Geometry: final body of the model. Coordinates: model frame, mm. A direction names the side the tool comes from. Round coordinates to 2 decimals unless told otherwise and drop trailing zeros. Loops run counter-clockwise (first coordinate to the right, second up) from the corner with the lowest first, then second, coordinate; pieces in that order, holes last. Notation, with made-up numbers: M -10,-8.75 L 14,-8.75 A21 cw 14,15.25 Z; hole C 82.5,67.5 d10. An arc over 180 degrees is marked long. Answer as a JSON object with one key per item and string values.
```python
from build123d import *

# Parameters (mm, degrees)
CHAMFER1_SIZE         = 1.2
M3_TAPPED_HOLE1_D     = 2.5
M3_TAPPED_HOLE1_DEPTH = 7.5
M3_TAPPED_HOLE1_TIP   = 0.751075774
CHAMFER2_SIZE         = 0.5


with BuildPart() as part:
    # Sketch1 → Revolve1 (revolve)
    with BuildSketch(Plane.XY, mode=Mode.PRIVATE) as revolve1_sk:
        Polygon((0, 0), (0, 3), (2.5, 3), (2.5, 5), (5, 5), (5, 3), (10, 3), (10, 2.9), (55.5, 2.9), (55.5, 3), (65.5, 3), (65.5, 0), align=None)
    revolve(revolve1_sk.sketch.rotate(Axis((0, 0, 0), (1, 0, 0)), 90), axis=Axis((0, 0, 0), (1, 0, 0)))

    # Chamfer1
    chamfer1_edges = [part.edges().sort_by_distance(p)[0] for p in [
        (5, 0, -5),
    ]]
    chamfer(chamfer1_edges, length=CHAMFER1_SIZE)

    # M3 Tapped Hole1
    with Locations(Plane.ZY):
        with Locations((0, 0)):
            Hole(M3_TAPPED_HOLE1_D / 2, depth=M3_TAPPED_HOLE1_DEPTH)
            with Locations((0, 0, -(M3_TAPPED_HOLE1_DEPTH + M3_TAPPED_HOLE1_TIP / 2))):  # 118° drill point
                Cone(0, M3_TAPPED_HOLE1_D / 2, M3_TAPPED_HOLE1_TIP, mode=Mode.SUBTRACT)

    # Chamfer2
    chamfer2_edges = [part.edges().sort_by_distance(p)[0] for p in [
        (0, 0, -3),
        (65.5, 0, -3),
    ]]
    chamfer(chamfer2_edges, length=CHAMFER2_SIZE)


solid = part.part
```
1) First-contact query: pin 1 (6 mm diameter, centred on x = 42, y = -1, fed in from +Z); pin 2 (2 mm diameter, centred on y = -0.5, z = -3.5, fed in from +X); pin 3 (2 mm diameter, centred on x = 8, z = -1.5, fed in from +Y). Flat tips, straight axial feed; report the tip coordinate or a pass-through.
Geometry results:
{"pin 1": "z = 2.9", "pin 2": "x = 65.46", "pin 3": "y = 2.96"}
2) Cut plane A-A on x = 26. Return the cut outline in (y, z), and give its area (3 significant figures).
Geometry results:
{"outline": "C 0,0 d5.8", "area": "26.4 mm2"}
3) Set-up query: faces 4 (the face through (60.32, -0.9, 2.86)), 5 (the face through (33.1, -0.1, -2.9)), 6 (the face through (1.51, -0.9, 2.86)), 7 (the face through (65.5, 0, 0)). Return all of +Z, -Z, +X, -X, +Y, -Y with unobstructed straight access to the full face (end or side cutting, diameter ignored); none if empty.
Geometry results:
{"face 4": "+X", "face 5": "none", "face 6": "-X", "face 7": "+Z, -Z, +X, +Y, -Y"}
4) Line query: probe 1 along Y at (x, z) = (1.75, 0); probe 2 along Y at (x, z) = (3.25, 0); probe 3 along X at (y, z) = (-3, 2). Output: solid intervals per line, ascending.
Geometry results:
{"probe 1": "-3 to -1.25, 1.25 to 3", "probe 2": "-5 to -1.25, 1.25 to 5", "probe 3": "2.5 to 5"}
5) Pull-direction query (Y, two-part tool) for faces 1 (the face through (3, 0, -5)), 2 (the face through (3.8, -1.22, 0.27)), 3 (the face through (0, -1, -1)); classes: +Y half, -Y half, draft (parallel to the pull), parting line (faces both ways), or undercut.
Geometry results:
{"face 1": "parting line", "face 2": "undercut", "face 3": "draft"}
